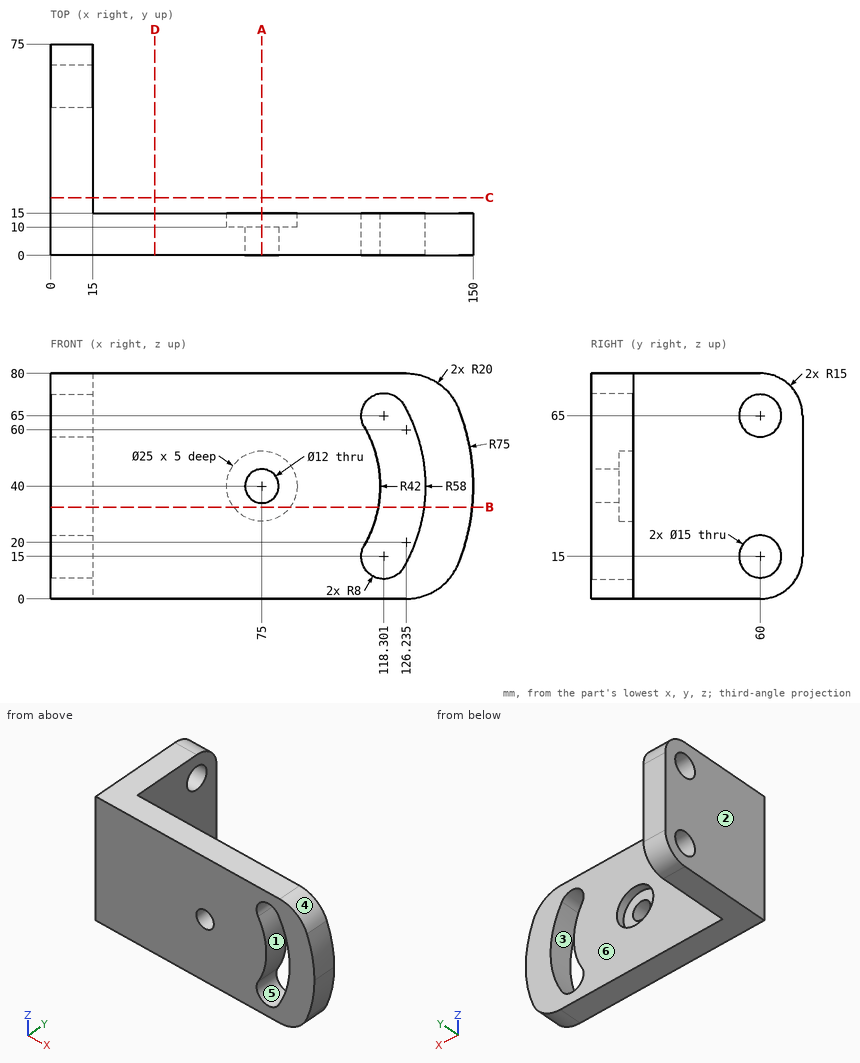
Here's the drawing with two shaded views (mm, measured from the low corner). I have some questions. A direction names the side the tool comes from. Round coordinates to 2 decimals unless told otherwise and drop trailing zeros. Order: outer loops, then holes, each group sorted by start corner. A loop starts at its lowest first (then second) coordinate and runs counter-clockwise, first axis right, second up. Notation, with made-up numbers: M 87.25,-5.5 L 117.25,-5.5 A13 ccw 117.25,17.5 Z; hole C 51,29 d7. An arc over 180 degrees is marked long. Use CSV: the item, a comma, the result in double quotes.
1) On a 3-axis mill with a long thin cutter (end or side, diameter ignored), from which of +Z, -Z, +X, -X, +Y, -Y can I reach the whole of each face in a straight line? I mean the marked faces 5 and 6. Say none if no direction works.
Taken from the geometry:
face 5,"+Y, -Y"
face 6,"+Z, -Z, +X, +Y"
2) I need wall thicknesses on line 1 along X through (y, z) = (2, 40); line 2 along X through (y, z) = (11.95, 40); line 3 along Z through (x, y) = (75, 14.05). Which ranges of each line are inside material? Lowest first, please. Write a range as [from, to].
Taken from the geometry:
line 1,"[0, 69], [81, 117], [133, 150]"
line 2,"[0, 62.5], [87.5, 117], [133, 150]"
line 3,"[0, 27.5], [52.5, 80]"
3) I want a section at C-C (y = 20.5). List the corners of the cut face in (x, z) for me, then the cut area to 3 significant figures.
Taken from the geometry:
outline,"M 0,0 L 15,0 L 15,80 L 0,80 Z"
area,"1,200 mm^2"
4) I want a section at B-B (z = 32.5). List the corners of the cut face in (x, y) for me (1 decimal), then the cut area to 3 significant figures.
Taken from the geometry:
outline,"M 0,0 L 116.3,0 L 116.3,15 L 85,15 L 85,10 L 65,10 L 65,15 L 15,15 L 15,75 L 0,75 Z; M 132.5,0 L 149.6,0 L 149.6,15 L 132.5,15 Z"
area,"2,800 mm^2"
5) I'm going to push flat-ended pins straight in: P1, Ø10, axis at y = 15, z = 56.5, coming from the +X side; P2, Ø17, axis at y = 60, z = 65, coming from the +X side; P3, Ø15.5, axis at x = 75, z = 40, coming from the +Y side. Where does each tip first touch, or does it pass through?
Taken from the geometry:
P1,"x = 149.11"
P2,"x = 15"
P3,"y = 10"
6) I want a section at A-A (x = 75). List the corners of the cut face in (y, z) for me, then the cut area to 3 significant figures.
Taken from the geometry:
outline,"M 0,0 L 15,0 L 15,27.5 L 10,27.5 L 10,34 L 0,34 Z; M 0,46 L 10,46 L 10,52.5 L 15,52.5 L 15,80 L 0,80 Z"
area,"955 mm^2"
7) If we mould it in two halves opening along Z, with no side actions, what happens to the marked faces 1, 2, 3 and 4? For each: pulls with the +Z half, pulls with the -Z half, needs draft (parallel to the pull), parting line crosses it, or undercut.
Taken from the geometry:
face 1,"undercut"
face 2,"needs draft"
face 3,"undercut"
face 4,"pulls with the +Z half"
